The listing builds one solid part. Answer for the finished solid, in the listing's coordinates (mm). A direction names the side the tool comes from. Round coordinates to 2 decimals unless told otherwise and drop trailing zeros. Write each loop counter-clockwise with the first axis right and the second up, starting at its lowest first coordinate (ties: lowest second). Pieces come first, ordered by that corner, then holes. Notation, with made-up numbers: M -27,-25.75 L 4,-25.75 A31 ccw 4,4.25 Z; hole C 6.25,11.5 d7. An arc over 180 degrees is marked long. One line per item, written item: value. Start each with the question number.
(1) Section B-B (z = -24.5) is taken. Determine the outline of the cut face in (x, y), plus the area to 3 significant figures.
(2) Consider probe 1 along X at (y, z) = (8.5, -37.5); probe 2 along Y at (x, z) = (-10.5, -41); probe 3 along Z at (x, y) = (-17.5, 39.5). Determine where each line is inside the solid, lowest interval first.
(3) Section D-D (y = 28) is taken. Determine the outline of the cut face in (x, z).
(4) For a pull along X with two mould halves and no side action, classify faces 6 (the flat face through (0, 9, 52.5)), 7 (the flat face through (5, 38, 23)), 8 (the cylindrical face through (-41.32, 9.13, 35.87)) as released by +X, released by -X, zero draft, split by the parting line, or undercut.
(5) Section C-C (x = -18) is taken. Determine the outline of the cut face in (y, z).
(6) For faces 1 (the flat face through (0, 73, -40)), 2 (the flat face through (-15, 53, 7.5)), 3 (the flat face through (24, 53, -6)), 4 (the cylindrical face through (3.604, 25.605, -16.054)), 5 (the flat face through (-24, 53, -6)), determine the directions among +Z, -Z, +X, -X, +Y, -Y from which every point of the face is accessible in a straight line to the end or side of a thin tool.
(7) Given P1, Ø15, axis at x = -17.5, y = 50, coming from the +Z side; P2, Ø8, axis at y = 33, z = 13, coming from the -X side; P3, Ø12, axis at x = 17.5, y = 52.5, coming from the -Z side, each flat-ended and moving along its own axis, determine where each tip first touches the part or whether it passes through.
(8) Section A-A (y = 16) is taken. Determine the outline of the cut face in (x, z), plus the area to 3 significant figures.
```python
from build123d import *

# Parameters (mm, degrees)
BASE_PLATE_DEPTH           = 18
MOUNTING_HOLES_SKETCH_R    = 7.5
MOUNTING_HOLES_4X_15_DEPTH = 18
UPRIGHT_COLUMN_SKETCH_W    = 48
UPRIGHT_COLUMN_SKETCH_H    = 70
UPRIGHT_COLUMN_DEPTH       = 7.5
SUPPORT_RIB_REACH          = 115.584
SUPPORT_RIB_SKETCH_WALL_W  = 312.383924088
SUPPORT_RIB_SKETCH_WALL_H  = 10
CLEVIS_LUG_1_SKETCH_R      = 12
CLEVIS_LUG_1_DEPTH         = 15
CLEVIS_START               = 15
CLEVIS_LUG_2_SKETCH_R      = 12
CLEVIS_LUG_2_DEPTH         = 15


with BuildPart() as part:
    # Base Plate Sketch → Base Plate (new body)
    with BuildSketch(Plane(origin=(0, 0, 0), x_dir=(1, 0, 0), z_dir=(0, 1, 0))):
        with BuildLine():
            Line((-34, -52.5), (34, -52.5))
            ThreePointArc((34, -52.5), (44.606601718, -48.106601718), (49, -37.5))
            Line((49, -37.5), (49, 37.5))
            ThreePointArc((49, 37.5), (44.606601718, 48.106601718), (34, 52.5))
            Line((34, 52.5), (-34, 52.5))
            ThreePointArc((-34, 52.5), (-44.606601718, 48.106601718), (-49, 37.5))
            Line((-49, 37.5), (-49, -37.5))
            ThreePointArc((-49, -37.5), (-44.606601718, -48.106601718), (-34, -52.5))
        make_face()
    extrude(amount=BASE_PLATE_DEPTH)

    # Mounting Holes Sketch → Mounting Holes 4xØ15 (cut)
    with BuildSketch(Plane(origin=(0, 18, 0), x_dir=(1, 0, 0), z_dir=(0, 1, 0))):
        with Locations(Location((-34, 37.5, 0), (0, 0, 270))):
            Circle(MOUNTING_HOLES_SKETCH_R)
        with Locations(Location((34, 37.5, 0), (0, 0, 270))):
            Circle(MOUNTING_HOLES_SKETCH_R)
        with Locations(Location((-34, -37.5, 0), (0, 0, 270))):
            Circle(MOUNTING_HOLES_SKETCH_R)
        with Locations(Location((34, -37.5, 0), (0, 0, 270))):
            Circle(MOUNTING_HOLES_SKETCH_R)
    extrude(amount=-MOUNTING_HOLES_4X_15_DEPTH, mode=Mode.SUBTRACT)

    # Upright Column Sketch → Upright Column (add, symmetric)
    with BuildSketch(Plane.XY):
        with Locations((0, 53)):
            Rectangle(UPRIGHT_COLUMN_SKETCH_W, UPRIGHT_COLUMN_SKETCH_H)
    extrude(amount=UPRIGHT_COLUMN_DEPTH, both=True)

    # Support Rib Sketch wall → Support Rib (add, up to next)
    with BuildSketch(Plane(origin=(0, 53, 30), x_dir=(0, -0.841178475377, 0.540757591313), z_dir=(0, -0.540757591313, -0.841178475377)), mode=Mode.PRIVATE) as support_rib_sk1:
        Rectangle(SUPPORT_RIB_SKETCH_WALL_W, SUPPORT_RIB_SKETCH_WALL_H)
    support_rib_tool1 = extrude(support_rib_sk1.sketch, amount=SUPPORT_RIB_REACH, mode=Mode.PRIVATE) - part.part
    add(support_rib_tool1.solids().sort_by_distance((0, 53, 30))[0])

    # Clevis Lug 1 Sketch → Clevis Lug 1 (add)
    with BuildSketch(Plane(origin=(0, 88, 0), x_dir=(1, 0, 0), z_dir=(0, 1, 0))):
        with BuildLine():
            Line((-24, -7.5), (-24, 27.5))
            ThreePointArc((-24, 27.5), (0, 51.5), (24, 27.5))
            Line((24, 27.5), (24, -7.5))
            Line((24, -7.5), (-24, -7.5))
        make_face()
        with Locations(Location((0, 27.5, 0), (0, 0, 270))):
            Circle(CLEVIS_LUG_1_SKETCH_R, mode=Mode.SUBTRACT)
    extrude(amount=-CLEVIS_LUG_1_DEPTH)

    # Clevis Lug 2 Sketch → Clevis Lug 2 (add)
    with BuildSketch(Plane(origin=(0, 18, 0), x_dir=(1, 0, 0), z_dir=(0, 1, 0)).offset(CLEVIS_START)):
        with BuildLine():
            Line((-24, 27.5), (-24, 7.5))
            Line((-24, 7.5), (24, 7.5))
            Line((24, 7.5), (24, 27.5))
            ThreePointArc((24, 27.5), (0, 51.5), (-24, 27.5))
        make_face()
        with Locations(Location((0, 27.5, 0), (0, 0, 270))):
            Circle(CLEVIS_LUG_2_SKETCH_R, mode=Mode.SUBTRACT)
    extrude(amount=-CLEVIS_LUG_2_DEPTH)


solid = part.part
```
Recorded:
1. outline: M -49,0 L 49,0 L 49,18 L 24,18 L 24,33 L 11.62,33 L 11.62,18 L -11.62,18 L -11.62,33 L -24,33 L -24,18 L -49,18 Z; M -24,73 L -11.62,73 L -11.62,88 L -24,88 Z; M 11.62,73 L 24,73 L 24,88 L 11.62,88 Z
1. area: 2,510 mm2
2. probe 1: x = -49 to -41.5, -26.5 to 26.5, 41.5 to 49
2. probe 2: y = 0 to 33, 73 to 88
2. probe 3: z = -7.5 to 7.5
3. outline: M -24,-27.5 A24 ccw 24,-27.5 L 24,7.5 L 5,7.5 L 5,46.07 L -5,46.07 L -5,7.5 L -24,7.5 Z; hole C 0,-27.5 d24
4. face 6: zero draft
4. face 7: released by +X
4. face 8: undercut
5. outline: M 0,-52.5 L 18,-52.5 L 18,-43.37 L 33,-43.37 L 33,-7.5 L 73,-7.5 L 73,-43.37 L 88,-43.37 L 88,7.5 L 18,7.5 L 18,52.5 L 0,52.5 Z
6. face 1: -Z, +X, -X
6. face 2: +Z, -X, +Y
6. face 3: +Z, -Z, +X, +Y
6. face 4: +Y
6. face 5: +Z, -Z, -X, +Y
7. P1: stops at z = 7.5
7. P2: stops at x = -5
7. P3: stops at z = -7.5
8. outline: M -49,-37.5 A15 ccw -34,-52.5 L 34,-52.5 A15 ccw 49,-37.5 L 49,37.5 A15 ccw 34,52.5 L -34,52.5 A15 ccw -49,37.5 Z; hole C -34,-37.5 d15; hole C -34,37.5 d15; hole C 34,-37.5 d15; hole C 34,37.5 d15
8. area: 9,390 mm2
